```python
from build123d import *

# Parameters (mm, degrees)
SKETCH_1_R          = 20
EXTRUDE_1_DEPTH     = 90
EXTRUDE_2_DEPTH     = 5
SKETCH_3_R          = 4
CUT_EXTRUDE_1_DEPTH = 60
CUT_EXTRUDE_2_DEPTH = 20


with BuildPart() as part:
    # Sketch 1 → Extrude 1 (new body)
    with BuildSketch(Plane.XY):
        with Locations(Location((0, 0, 0), (0, 0, 180))):
            Circle(SKETCH_1_R)
    extrude(amount=EXTRUDE_1_DEPTH)

    # Sketch 2 → Extrude 2 (add)
    with BuildSketch(Plane.XY.offset(90)):
        with BuildLine():
            Line((-43.90625, 11.873971995), (-7.8125, 23.74794399))
            ThreePointArc((-7.8125, 23.74794399), (25, 0), (-7.8125, -23.74794399))
            Line((-7.8125, -23.74794399), (-43.90625, -11.873971995))
            ThreePointArc((-43.90625, -11.873971995), (-52.5, 0), (-43.90625, 11.873971995))
        make_face()
    extrude(amount=-EXTRUDE_2_DEPTH)

    # Sketch 3 → Cut-Extrude 1 (cut)
    with BuildSketch(Plane.XY.offset(90)):
        Circle(SKETCH_3_R)
    extrude(amount=-CUT_EXTRUDE_1_DEPTH, mode=Mode.SUBTRACT)

    # Sketch 4 → Cut-Extrude 2 (cut)
    with BuildSketch(Plane(origin=(0, 0, 0), x_dir=(1, 0, 0), z_dir=(0, 1, 0))):
        with BuildLine():
            ThreePointArc((4, -42.5), (2.828427125, -39.671572875), (0, -38.5))
            Line((0, -38.5), (0, -46.5))
            ThreePointArc((0, -46.5), (2.828427125, -45.328427125), (4, -42.5))
        make_face()
        with BuildLine():
            Line((0, -46.5), (0, -38.5))
            ThreePointArc((0, -38.5), (-4, -42.5), (0, -46.5))
        make_face()
    extrude(amount=-CUT_EXTRUDE_2_DEPTH, mode=Mode.SUBTRACT)


solid = part.part
```
Work out the finished part from the listing and answer in its coordinate system (mm). A direction names the side the tool comes from. Round coordinates to 2 decimals unless told otherwise and drop trailing zeros. Order: outer loops, then holes, each group sorted by start corner. A loop starts at its lowest first (then second) coordinate and runs counter-clockwise, first axis right, second up.
Q1. A cutting plane is placed at A-A, the plane x = 2. Determine the outline of the cut face in (y, z), then the cut area to 3 significant figures.
Solution:
outline: (-24.92, 85) - (-19.9, 85) - (-19.9, 45.96) - (-3.46, 45.96) - (-3.46, 90) - (-24.92, 90) - close; (-19.9, 0) - (19.9, 0) - (19.9, 85) - (24.92, 85) - (24.92, 90) - (3.46, 90) - (3.46, 30) - (-3.46, 30) - (-3.46, 39.04) - (-19.9, 39.04) - close
area: 3,100 mm2
Q2. A tool of negligible diameter and unlimited length cuts with its end or side. For faces 1 (the cylindrical face through (2.15, 3.373, 60.42)), 2 (the cylindrical face through (4.336, 19.524, 41.905)), 3 (the cylindrical face through (24.99, 0.66, 87.54)), from which of +Z, -Z, +X, -X, +Y, -Y can it reach the whole face along a straight path? Write none if from no direction.
Solution:
face 1: +Z
face 2: -Z
face 3: +Z, -Z
Q3. Given pin 1 Ø3 at (x, z) = (3, 68.5) entering from +Y; pin 2 Ø8 at (x, z) = (-26.5, 77.5) entering from -Y; pin 3 Ø10 at (y, z) = (20, 79.5) entering from -X; pin 4 Ø10 at (x, z) = (6, 64) entering from -Y (3 decimals), each flat-ended and moving along its own axis, determine where each tip first touches the part or whether it passes through.
Solution:
pin 1: stops at y = 19.94
pin 2: passes through
pin 3: stops at x = -13.23
pin 4: stops at y = -19.975
Q4. A cutting plane is placed at B-B, the plane x = -6. Determine the outline of the cut face in (y, z), then the cut area to 3 significant figures.
Solution:
outline: (-24.27, 85) - (-19.08, 85) - (-19.08, 0) - (19.08, 0) - (19.08, 85) - (24.27, 85) - (24.27, 90) - (-24.27, 90) - close
area: 3,490 mm2
Q5. The mould has two halves that part along X. Classify faces 4 (the flat face through (0, 0, 30)), 5 (the flat face through (0, 0, 0)), 6 (the cylindrical face through (-52.5, -0.2, 87.5)): pulls with the +X half, pulls with the -X half, needs draft (parallel to the pull), parting line crosses it, or undercut.
Solution:
face 4: undercut
face 5: needs draft
face 6: pulls with the -X half
Q6. Find the intervals of material crossed by line 1 along Z through (x, y) = (-3, 20); line 2 along Y through (x, z) = (0, 64); line 3 along X through (y, z) = (-2, 77.5), in increasing order.
Solution:
line 1: z = 85 to 90
line 2: y = -20 to -4, 4 to 20
line 3: x = -19.9 to -3.46, 3.46 to 19.9
Q7. A cutting plane is placed at C-C, the plane z = 65. Determine the outline of the cut face in (x, y).
Solution:
outline: circle Ø40 at (0, 0); hole circle Ø8 at (0, 0)
Q8. A cutting plane is placed at D-D, the plane y = 16. Determine the outline of the cut face in (x, z), then the cut area to 3 significant figures.
Solution:
outline: (-31.36, 85) - (-12, 85) - (-12, 0) - (12, 0) - (12, 85) - (19.21, 85) - (19.21, 90) - (-31.36, 90) - close
area: 2,290 mm2
